from build123d import *
from OCP.BRepFilletAPI import BRepFilletAPI_MakeChamfer

# Parameters (mm, degrees)
EXTRUDE_1_DEPTH = 69
CHAMFER_1_SIZE  = 20
SKETCH_3_R      = 30
EXTRUDE_2_DEPTH = 18
CHAMFER_2_SIZE  = 20
CHAMFER_2_SIZE2 = 14.142135624


with BuildPart() as part:
    # 草图1 → 凸台-拉伸1 (new body)
    with BuildSketch(Plane.XY):
        Polygon((0, 0), (0, -90), (90, -90), align=None)
    extrude(amount=EXTRUDE_1_DEPTH)

    # 倒角1
    chamfer_1_edges = [part.edges().sort_by_distance(p)[0] for p in [
        (0, -90, 34.5),
    ]]
    chamfer(chamfer_1_edges, length=CHAMFER_1_SIZE)

    # 草图3 → 凸台-拉伸2 (add)
    with BuildSketch(Plane(origin=(0, 0, 0), x_dir=(0, 0, -1), z_dir=(0.7071067811865475, 0.7071067811865476, 0))):
        with Locations(Location((-34.5, -63.639610307, 0), (0, 0, 90))):
            Circle(SKETCH_3_R)
    extrude(amount=EXTRUDE_2_DEPTH)

    # 倒角2: one chamfer whose edges measure the first distance from different faces: ONE call of the kernel's chamfer builder (chamfer() names one face for all edges)
    chamfer_2_edges_1 = [part.edges().sort_by_distance(p)[0] for p in [
        (90, -90, 34.5),
    ]]
    chamfer_2_side_1 = [part.faces().sort_by_distance(p)[0] for p in [
        (55, -90, 34.5),
    ]]
    chamfer_2_edges_2 = [part.edges().sort_by_distance(p)[0] for p in [
        (0, 0, 34.5),
    ]]
    chamfer_2_side_2 = [part.faces().sort_by_distance(p)[0] for p in [
        (88.976256868, -88.976256868, 34.5),
    ]]
    chamfer_2 = BRepFilletAPI_MakeChamfer(part.part.solid().wrapped)
    for e in chamfer_2_edges_1:
        chamfer_2.Add(CHAMFER_2_SIZE, CHAMFER_2_SIZE2, e.wrapped, chamfer_2_side_1[0].wrapped)  # the first distance lies on this face
    for e in chamfer_2_edges_2:
        chamfer_2.Add(CHAMFER_2_SIZE, CHAMFER_2_SIZE2, e.wrapped, chamfer_2_side_2[0].wrapped)  # the first distance lies on this face
    add(Compound.cast(chamfer_2.Shape()), mode=Mode.REPLACE)


solid = part.part
Geometry check sheet. Reference: the model listing, model coordinates, mm. A direction names the side the tool comes from. Give positions to 0.01 mm unless a question says otherwise; leave off trailing zeros. Write each loop counter-clockwise with the first axis right and the second up, starting at its lowest first coordinate (ties: lowest second). Pieces come first, ordered by that corner, then holes.
1) Cross-section at C-C (z = 23). Record the boundary of the cut face in (x, y).
Values follow:
outline: (0, -70) - (20, -90) - (70, -90) - (80, -80) - (64.59, -64.59) - (77.32, -51.86) - (38.14, -12.68) - (25.41, -25.41) - (14.14, -14.14) - (0, -14.14) - close
2) Thickness scan on line 1 (X direction, y = -27, z = 54.5); line 2 (Y direction, x = 71, z = 47.5); line 3 (Y direction, x = 49, z = 61). Record the ranges inside material, lowest first.
Values follow:
line 1: x = 0 to 27, 31.38 to 52.46
line 2: y = -89 to -71, -57.24 to -45.54
line 3: y = -90 to -23.54
3) Cross-section at B-B (x = 16.5). Record the boundary of the cut face in (y, z).
Values follow:
outline: (-86.5, 0) - (-16.5, 0) - (-16.5, 69) - (-86.5, 69) - close
4) Release check for a two-part mould opening along X. For faces 3 (the face through (75, -85, 34)), 4 (the face through (69, -69, 34)), 5 (the face through (0, -42, 34)) record: released by +X, released by -X, zero draft, split by the parting line, or undercut.
Values follow:
face 3: released by +X
face 4: undercut
face 5: released by -X
5) Go/stop test with flat-tipped pins: pin 1 Ø4 at (x, y) = (12.5, -72) entering from -Z; pin 2 Ø3 at (x, z) = (49, 13.5) entering from +Y; pin 3 Ø1 at (x, z) = (17.5, 8) entering from -Y; pin 4 Ø15.5 at (x, z) = (7.5, 24.5) entering from +Y. Record where each tip stops, or that it passes through.
Values follow:
pin 1: stops at z = 0
pin 2: stops at y = -22.04
pin 3: stops at y = -88
pin 4: stops at y = -14.14
6) Set-up check for faces 1 (the face through (7, -14.142, 34)), 2 (the face through (31, -60, 0)): record each of +Z, -Z, +X, -X, +Y, -Y from which the full face is reachable in a straight line by a thin tool's end or side.
Values follow:
face 1: +Z, -Z, -X, +Y
face 2: -Z, +X, -X, +Y, -Y
7) Cross-section at A-A (z = 39). Record the boundary of the cut face in (x, y), plus the area to 3 significant figures.
Values follow:
outline: (0, -70) - (20, -90) - (70, -90) - (80, -80) - (65.97, -65.97) - (78.7, -53.25) - (36.75, -11.3) - (24.03, -24.03) - (14.14, -14.14) - (0, -14.14) - close
area: 4,720 mm2
